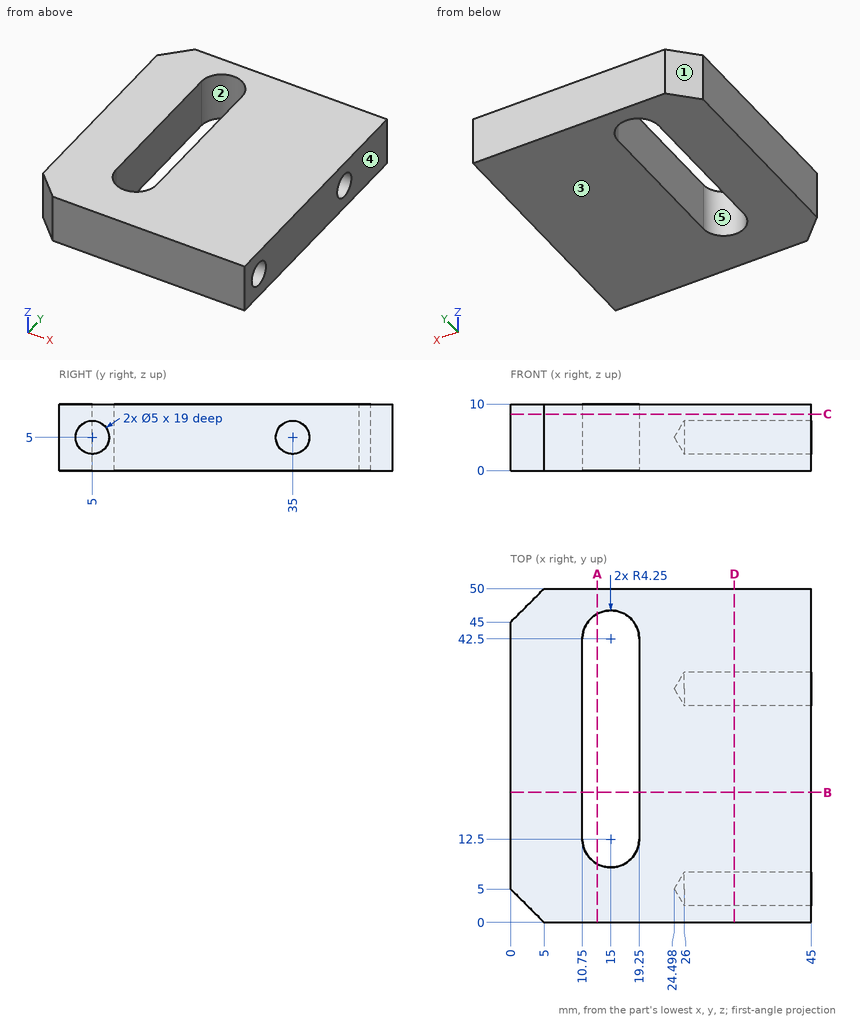
Input: dimensioned drawing with shaded views. Units: mm. Origin: part minimum x, y, z. A direction names the side the tool comes from. Coordinates: 2 decimals unless noted, no trailing zeros. Order: outer loops, then holes, each group sorted by start corner. A loop starts at its lowest first (then second) coordinate and runs counter-clockwise, first axis right, second up. Notation, with made-up numbers: (12.5, 27) -> (62.5, 27) arc R26 cw to (62.5, 43) -> close; hole circle Ø10 at (88.5, 76.25). An arc over 180 degrees is marked (long way). Answer in a Markdown table with one row per item.
Item 1: Section D-D on x = 33.5. Output: boundary loops of the cut face in (y, z).
Return value:
| item | result |
|---|---|
| outline | (0, 0) -> (50, 0) -> (50, 10) -> (0, 10) -> close; hole circle Ø5 at (5, 5); hole circle Ø5 at (35, 5) |
Item 2: Ray query, L1, parallel to Y at x = 35.5, z = 5.25; L2, parallel to Z at x = 39, y = 35; L3, parallel to Y at x = 15, z = 9.75. Return the intervals inside material, ascending.
Return value:
| item | result |
|---|---|
| L1 | y = 0 to 2.51, 7.49 to 32.51, 37.49 to 50 |
| L2 | z = 0 to 2.5, 7.5 to 10 |
| L3 | y = 0 to 8.25, 46.75 to 50 |
Item 3: Access query for the marked faces 4 and 5. Directions: +Z, -Z, +X, -X, +Y, -Y. A direction counts if a zero-diameter tool reaches every point of the face in a straight line with its end or side. Return the directions, or none.
Return value:
| item | result |
|---|---|
| face 4 | +Z, -Z, +X, +Y, -Y |
| face 5 | +Z, -Z |
Item 4: Section A-A on x = 13. Output: boundary loops of the cut face in (y, z), plus the area to 3 significant figures.
Return value:
| item | result |
|---|---|
| outline | (0, 0) -> (8.75, 0) -> (8.75, 10) -> (0, 10) -> close; (46.25, 0) -> (50, 0) -> (50, 10) -> (46.25, 10) -> close |
| area | 125 mm² |
Item 5: Section C-C on z = 8.5. Output: boundary loops of the cut face in (x, y), plus the area to 3 significant figures.
Return value:
| item | result |
|---|---|
| outline | (0, 5) -> (5, 0) -> (45, 0) -> (45, 50) -> (5, 50) -> (0, 45) -> close; hole (10.75, 12.5) arc R4.25 ccw to (19.25, 12.5) -> (19.25, 42.5) arc R4.25 ccw to (10.75, 42.5) -> close |
| area | 1,910 mm² |
Item 6: Section B-B on y = 19.5. Output: boundary loops of the cut face in (x, z).
Return value:
| item | result |
|---|---|
| outline | (0, 0) -> (10.75, 0) -> (10.75, 10) -> (0, 10) -> close; (19.25, 0) -> (45, 0) -> (45, 10) -> (19.25, 10) -> close |
Item 7: Draft query along Y for the marked faces 1, 2 and 3. Return one class per face: released by +Y, released by -Y, zero draft, split by the parting line, or undercut.
Return value:
| item | result |
|---|---|
| face 1 | released by +Y |
| face 2 | undercut |
| face 3 | zero draft |
Item 8: Contact query for a flat-ended pin moving along its axis: P1, Ø3, axis at y = 5, z = 5, coming from the -X side. Output: stop coordinate, or through.
Return value:
| item | result |
|---|---|
| P1 | stops at x = 0 |
